Geometry check sheet. Reference: the model listing, model coordinates, mm. Round coordinates to 2 decimals unless told otherwise and drop trailing zeros.
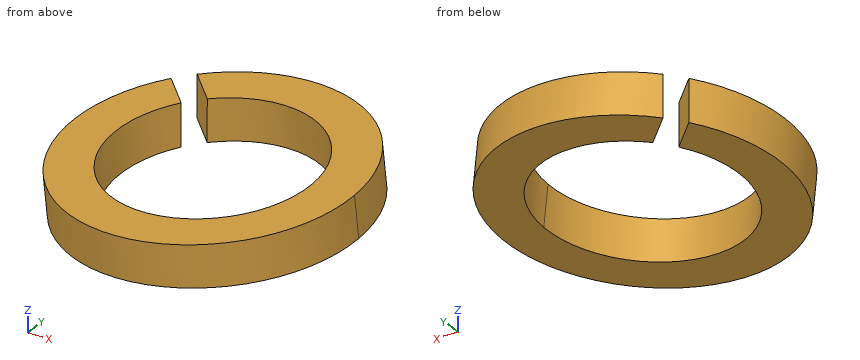
```python
from build123d import *

# Parameters (mm, degrees)
BASE_EXTRUDE_DEPTH      = 0.001
BASE_EXTRUDE_DEPTH_BACK = 0.001
SKETCH6_W               = 2.905
SKETCH6_H               = 3.96
SKETCH8_R               = 10.003955179
SKETCH8_R_2             = 7
BOSS_EXTRUDE1_DEPTH     = 2.945
CUT_EXTRUDE1_DEPTH      = 15.963360846
CUT_EXTRUDE1_DEPTH_BACK = 15.963360846


with BuildPart() as part:
    # Sketch6 → Base-Extrude (new, two sides: drawn at the far end of the back side and taken through both)
    with BuildSketch(Plane(origin=(-4.242640687, 4.242640687, 3.255), x_dir=(0.060826394912022484, 0.060826394912020985, -0.9962932797946665), z_dir=(0.7044857341934017, 0.7044857341933883, 0.08602151263484296)).offset(-BASE_EXTRUDE_DEPTH_BACK)):
        with Locations((1.4725, 2)):
            Rectangle(SKETCH6_W, SKETCH6_H)
    extrude(amount=BASE_EXTRUDE_DEPTH + BASE_EXTRUDE_DEPTH_BACK)

    # Sketch8 → Boss-Extrude1 (add)
    with BuildSketch(Plane(origin=(-0.196039494, -0.196039494, 3.210988109), x_dir=(0.9981483386916642, -0.003915635910269119, 0.06070059112141398), z_dir=(-0.060826394912022415, -0.0608263949120211, 0.9962932797946664))):
        with Locations(Location((0, 0, 0), (0, 0, 0.224766173))):
            Circle(SKETCH8_R)
        with Locations(Location((0, 0, 0), (0, 0, 0.224766173))):
            Circle(SKETCH8_R_2, mode=Mode.SUBTRACT)
    extrude(amount=-BOSS_EXTRUDE1_DEPTH)

    # Sketch9 → Cut-Extrude1 (cut, two sides: drawn at the far end of the back side and taken through both)
    with BuildSketch(Plane.XY.offset(-CUT_EXTRUDE1_DEPTH_BACK)):
        Polygon((-34.702943681, 35.798959192), (0.298841987, 0.797173523), (-0.797173523, -0.298841987), (-36.894974703, 35.798959192), align=None)
    extrude(amount=CUT_EXTRUDE1_DEPTH + CUT_EXTRUDE1_DEPTH_BACK, mode=Mode.SUBTRACT)


solid = part.part
```
(1) Sectioned sample at A-A, the plane y = 5.75. Give the number of separate pieces and of enclosed holes in the cut face, and give its area (3 significant figures).
Returned:
separate pieces: 3
enclosed holes: 0
area: 18.8 mm2
(2) Depth check by flat-ended pin: P1, Ø1.5, axis at x = 5, z = 2, coming from the +Y side; P2, Ø4, axis at x = 2, y = 8, coming from the +Z side; P3, Ø1.5, axis at x = -7, z = 2, coming from the +Y side. Enter the tip coordinate at first touch or a pass-through.
Returned:
P1: stops at y = 8.92
P2: stops at z = 4.01
P3: stops at y = 7.79
(3) Material ranges on line 1 (X direction, y = -1.25, z = 2.3); line 2 (Y direction, x = 6, z = 1.75); line 3 (Y direction, x = -3, z = 0.35), recorded low to high.
Returned:
line 1: x = -10.11 to -7.07, 6.78 to 9.82
line 2: y = -8.03 to -3.53, 3.36 to 7.86
line 3: y = -9.6 to -6.38
